Geometry check sheet. Reference: the model listing, model coordinates, mm. Face numbers are marked on the shaded views. A direction names the side the tool comes from. Round coordinates to 2 decimals unless told otherwise and drop trailing zeros. Write each loop counter-clockwise with the first axis right and the second up, starting at its lowest first coordinate (ties: lowest second). Pieces come first, ordered by that corner, then holes. Notation, with made-up numbers: (52, 14) - (105, 14) arc R7 cw to (105, 24) - close; hole circle Ø9 at (57, 73). An arc over 180 degrees is marked (long way). Return JSON: item names as keys, results as strings.
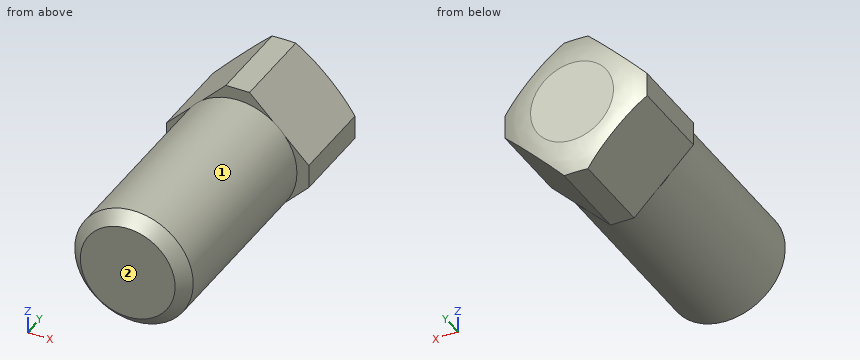
```python
from build123d import *

# Parameters (mm, degrees)
CHAMFER1_SIZE       = 1
SKETCH2_R           = 11.978178672
CUT_EXTRUDE2_DEPTH  = 8
SKETCH4_R           = 5
BOSS_EXTRUDE1_DEPTH = 1.5
CHAMFER2_SIZE       = 1


with BuildPart() as part:
    # Sketch1 → Revolve1 (revolve)
    with BuildSketch(Plane.XY, mode=Mode.PRIVATE) as revolve1_sk:
        Polygon((0, 0), (0, 24), (10, 24), (10, 16), (5, 16), (5, 0), align=None)
    revolve(revolve1_sk.sketch.rotate(Axis((0, 0, 0), (0, 1, 0)), 90), axis=Axis((0, 0, 0), (0, 1, 0)))

    # Chamfer1
    chamfer1_edges = [part.edges().sort_by_distance(p)[0] for p in [
        (0, 0, 5),
    ]]
    chamfer(chamfer1_edges, length=CHAMFER1_SIZE)

    # Sketch2 → Cut-Extrude2 (cut)
    with BuildSketch(Plane(origin=(0, 24, 0), x_dir=(1, 0, 0), z_dir=(0, 1, 0))):
        Circle(SKETCH2_R)
        Polygon((-1, 6), (1, 6), (6, 1), (6, -1), (1, -6), (-1, -6), (-6, -1), (-6, 1), align=None, mode=Mode.SUBTRACT)
    extrude(amount=-CUT_EXTRUDE2_DEPTH, mode=Mode.SUBTRACT)

    # Sketch3 → Cut-Revolve1 (revolve, cut)
    with BuildSketch(Plane.XY, mode=Mode.PRIVATE) as cut_revolve1_sk:
        with BuildLine():
            Line((3.5, 24), (5.57579334, 25.302795294))
            Line((5.57579334, 25.302795294), (6.462708925, 23.688216178))
            Line((6.462708925, 23.688216178), (6.758347453, 22.996814774))
            ThreePointArc((6.758347453, 22.996814774), (5.187612361, 23.688216178), (3.5, 24))
        make_face()
    revolve(cut_revolve1_sk.sketch.rotate(Axis((0, 0, 0), (0, 1, 0)), 90), axis=Axis((0, 0, 0), (0, 1, 0)), mode=Mode.SUBTRACT)

    # Sketch4 → Boss-Extrude1 (add, symmetric)
    with BuildSketch(Plane.XZ):
        with Locations(Location((0, 0, 0), (0, 0, 270))):
            Circle(SKETCH4_R)
    extrude(amount=BOSS_EXTRUDE1_DEPTH, both=True)

    # Chamfer2
    chamfer2_edges = [part.edges().sort_by_distance(p)[0] for p in [
        (0, -1.5, 5),
    ]]
    chamfer(chamfer2_edges, length=CHAMFER2_SIZE)


solid = part.part
```
(1) Access from +Z, -Z, +X, -X, +Y, -Y to the whole of each face (thin tool, end or side, straight path). Record for the marked faces 1 and 2.
Response values:
{"face 1": "-Y", "face 2": "+Z, -Z, +X, -X, -Y"}
(2) Section check A-A, the plane y = 20.5. Enter the section's corners in (x, z).
Response values:
{"outline": "(-6, -1) - (-1, -6) - (1, -6) - (6, -1) - (6, 1) - (1, 6) - (-1, 6) - (-6, 1) - close"}
(3) Gauge pin test, flat ends, axial feed: pin 1 (6 mm diameter, centred on y = 20.5, z = -3.5, fed in from -X); pin 2 (2 mm diameter, centred on x = 1, z = 5.5, fed in from -Y); pin 3 (2 mm diameter, centred on x = -4, y = 6, fed in from -Z); pin 4 (1 mm diameter, centred on x = -1, y = 7, fed in from -Z). Record the tip position at first contact, or that the pin passes through.
Response values:
{"pin 1": "stops at x = -6", "pin 2": "stops at y = -0.91", "pin 3": "stops at z = -4", "pin 4": "stops at z = -4.97"}
(4) Section check B-B, the plane y = 5.5. Enter the section's corners in (x, z), plus the area to 3 significant figures.
Response values:
{"outline": "circle Ø10 at (0, 0)", "area": "78.5 mm^2"}
(5) Material ranges on line 1 along Z through (x, y) = (-3, 12.25); line 2 along X through (y, z) = (22.5, -3.5), recorded low to high. Write a range as [from, to].
Response values:
{"line 1": "z = [-4, 4]", "line 2": "x = [-3.5, 3.5]"}
